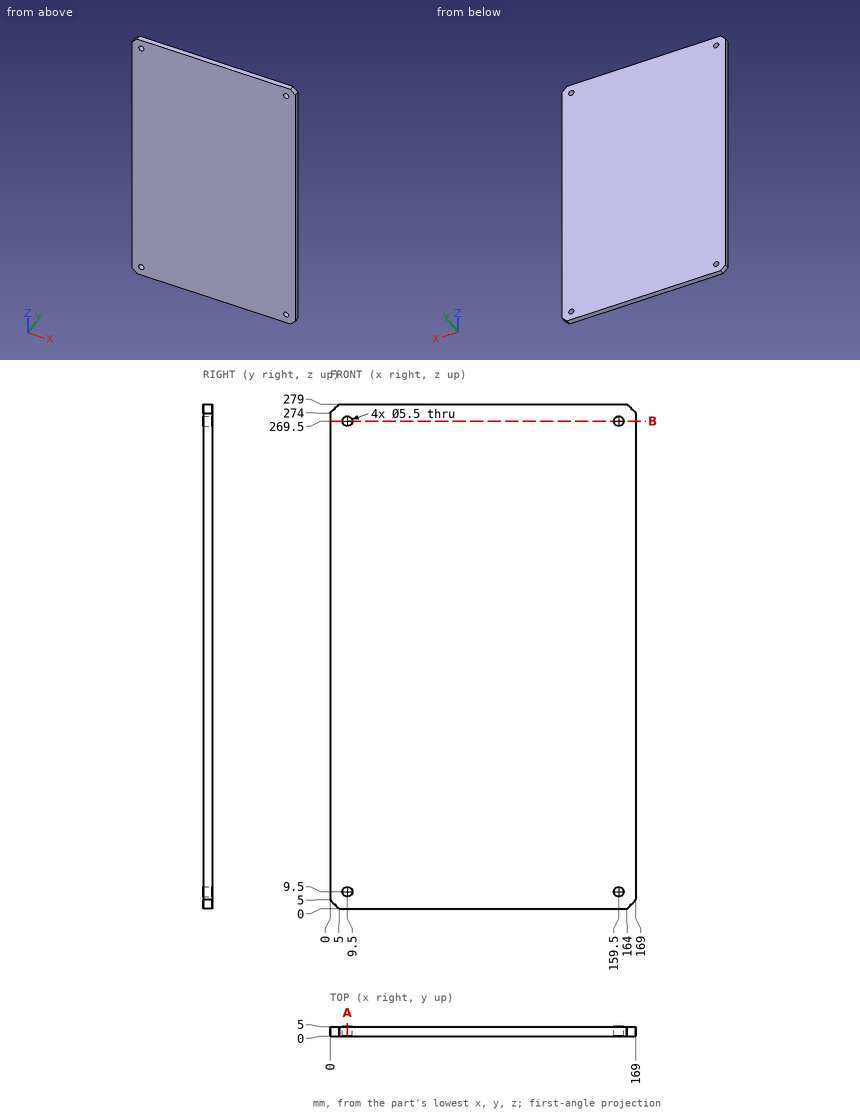
Could you check a few things on this drawing? It's one solid part, dimensions in mm from its lowest x, y, z. Coordinates: 2 decimals unless noted, no trailing zeros. Write each loop counter-clockwise with the first axis right and the second up, starting at its lowest first coordinate (ties: lowest second). Pieces come first, ordered by that corner, then holes. Notation, with made-up numbers: (71, -5.5) - (80, -5.5) arc R22 cw to (80, 29.5) - close; hole circle Ø1 at (77.25, 39.25). An arc over 180 degrees is marked (long way). Return JSON: item names as keys, results as strings. Group by question number.
Item 1: If we section it at B-B (z = 269.5): Write out the boundary of the cut face in (x, y), then the cut area to 3 significant figures.
Item 2: I'm going to push flat-ended pins straight in: pin 1 Ø2 at (x, y) = (120.5, 4) entering from -Z; pin 2 Ø5 at (x, z) = (9.5, 269.5) entering from -Y. Where does each tip first touch, or does it pass through?
Item 3: Please list where these lines run through material, in increasing order: probe 1 along X at (y, z) = (3.1, 9.5); probe 2 along Z at (x, y) = (159.5, 3.5).
Item 4: If we section it at A-A (x = 9.5): Write out the boundary of the cut face in (y, z), then the cut area to 3 significant figures.
Return value:
{
 "1": {"outline": "(0, 0) - (6.75, 0) - (6.75, 5) - (0, 5) - close; (12.25, 0) - (156.75, 0) - (156.75, 5) - (12.25, 5) - close; (162.25, 0) - (169, 0) - (169, 5) - (162.25, 5) - close", "area": "790 mm^2"},
 "2": {"pin 1": "stops at z = 0", "pin 2": "passes through"},
 "3": {"probe 1": "x = 0 to 6.75, 12.25 to 156.75, 162.25 to 169", "probe 2": "z = 0 to 6.75, 12.25 to 266.75, 272.25 to 279"},
 "4": {"outline": "(0, 0) - (5, 0) - (5, 6.75) - (0, 6.75) - close; (0, 12.25) - (5, 12.25) - (5, 266.75) - (0, 266.75) - close; (0, 272.25) - (5, 272.25) - (5, 279) - (0, 279) - close", "area": "1,340 mm^2"}
}
